from build123d import *

# Parameters (mm, degrees)
SKETCH1_R           = 2.3
BOSS_EXTRUDE1_DEPTH = 3
SKETCH3_W           = 2.8
SKETCH3_H           = 10
CUT_EXTRUDE1_DEPTH  = 10
SKETCH4_W           = 30
SKETCH4_H           = 3
BOSS_EXTRUDE2_DEPTH = 5


with BuildPart() as part:
    # Sketch1 → Boss-Extrude1 (new body)
    with BuildSketch(Plane.XY):
        Polygon((0, 0), (8, 0), (8, -22), (51, -22), (51, 0), (59, 0), (59, -36), (0, -36), align=None)
        with Locations((4.5, -15.05)):
            Circle(SKETCH1_R, mode=Mode.SUBTRACT)
        with Locations((4.5, -4.95)):
            Circle(SKETCH1_R, mode=Mode.SUBTRACT)
        with Locations((54.5, -4.95)):
            Circle(SKETCH1_R, mode=Mode.SUBTRACT)
        with Locations((54.5, -15.05)):
            Circle(SKETCH1_R, mode=Mode.SUBTRACT)
    extrude(amount=BOSS_EXTRUDE1_DEPTH)

    # Sketch3 → Cut-Extrude1 (cut)
    with BuildSketch(Plane.XY.offset(3)):
        with Locations((4, -27)):
            Rectangle(SKETCH3_W, SKETCH3_H)
        with Locations((55, -27)):
            Rectangle(SKETCH3_W, SKETCH3_H)
    extrude(amount=-CUT_EXTRUDE1_DEPTH, mode=Mode.SUBTRACT)

    # Sketch4 → Boss-Extrude2 (add)
    with BuildSketch(Plane.XZ.offset(36)):
        with Locations((29.5, 1.5)):
            Rectangle(SKETCH4_W, SKETCH4_H)
    extrude(amount=BOSS_EXTRUDE2_DEPTH)


solid = part.part
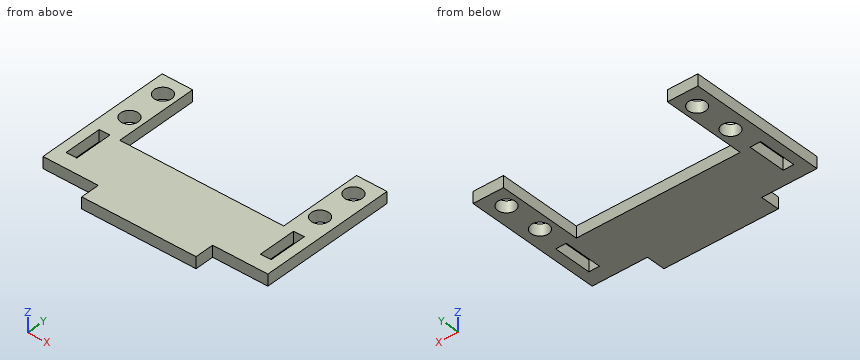
CAD build for the part. Positions are in the model's coordinates, mm. Round coordinates to 2 decimals unless told otherwise and drop trailing zeros. Order: outer loops, then holes, each group sorted by start corner. A loop starts at its lowest first (then second) coordinate and runs counter-clockwise, first axis right, second up. Notation, with made-up numbers: (3.25, 17) -> (54.25, 17) arc R18 cw to (54.25, 34) -> close; hole circle Ø2 at (-39.5, 1.25). An arc over 180 degrees is marked (long way). Write each question's results on one line, items separated by ' | '.
1. Cut at D-D (y = -26). Give the cut face in (x, z), plus the area to 3 significant figures.
Findings below:
outline: (0, 0) -> (2.6, 0) -> (2.6, 3) -> (0, 3) -> close; (5.4, 0) -> (53.6, 0) -> (53.6, 3) -> (5.4, 3) -> close; (56.4, 0) -> (59, 0) -> (59, 3) -> (56.4, 3) -> close | area: 160 mm²
2. Cut at A-A (y = -15.05). Give the cut face in (x, z), plus the area to 3 significant figures.
Findings below:
outline: (0, 0) -> (2.2, 0) -> (2.2, 3) -> (0, 3) -> close; (6.8, 0) -> (8, 0) -> (8, 3) -> (6.8, 3) -> close; (51, 0) -> (52.2, 0) -> (52.2, 3) -> (51, 3) -> close; (56.8, 0) -> (59, 0) -> (59, 3) -> (56.8, 3) -> close | area: 20.4 mm²
3. Flat gauge pins, fed straight in: P1, Ø1.5, axis at x = 53.5, z = 2, coming from the -Y side; P2, Ø1.5, axis at y = -39, z = 2, coming from the +X side; P3, Ø3, axis at x = 54.5, y = -4.95, coming from the -Z side. Where does each tip first touch, or does it go through?
Findings below:
P1: stops at y = -36 | P2: stops at x = 44.5 | P3: passes through
4. Wall check: line 1 along Y through (x, z) = (54.5, 1.8); line 2 along X through (y, z) = (-23, 1.35); line 3 along X through (y, z) = (-20.5, 1.7). Give the ranges that are in metal, low to high. Write a range as [from, to].
Findings below:
line 1: y = [-36, -32], [-22, -17.35], [-12.75, -7.25], [-2.65, 0] | line 2: x = [0, 2.6], [5.4, 53.6], [56.4, 59] | line 3: x = [0, 8], [51, 59]
5. Cut at C-C (x = 4.5). Give the cut face in (y, z), plus the area to 3 significant figures.
Findings below:
outline: (-36, 0) -> (-32, 0) -> (-32, 3) -> (-36, 3) -> close; (-22, 0) -> (-17.35, 0) -> (-17.35, 3) -> (-22, 3) -> close; (-12.75, 0) -> (-7.25, 0) -> (-7.25, 3) -> (-12.75, 3) -> close; (-2.65, 0) -> (0, 0) -> (0, 3) -> (-2.65, 3) -> close | area: 50.4 mm²
6. Cut at B-B (z = 0.5). Give the cut face in (x, y).
Findings below:
outline: (0, -36) -> (14.5, -36) -> (14.5, -41) -> (44.5, -41) -> (44.5, -36) -> (59, -36) -> (59, 0) -> (51, 0) -> (51, -22) -> (8, -22) -> (8, 0) -> (0, 0) -> close; hole circle Ø4.6 at (4.5, -15.05); hole circle Ø4.6 at (4.5, -4.95); hole (2.6, -32) -> (5.4, -32) -> (5.4, -22) -> (2.6, -22) -> close; hole circle Ø4.6 at (54.5, -15.05); hole circle Ø4.6 at (54.5, -4.95); hole (53.6, -32) -> (56.4, -32) -> (56.4, -22) -> (53.6, -22) -> close
